Study the drawing (mm; zero at the part's minimum x, y, z) and answer. A direction names the side the tool comes from. Coordinates: 2 decimals unless noted, no trailing zeros. Order: outer loops, then holes, each group sorted by start corner. A loop starts at its lowest first (then second) coordinate and runs counter-clockwise, first axis right, second up. Notation, with made-up numbers: (53, 31.5) -> (90, 31.5) arc R21 cw to (90, 51.5) -> close; hole circle Ø11 at (69.25, 58). An arc over 180 degrees is marked (long way). Put each result on its own line as item: value. Start each with the question number.
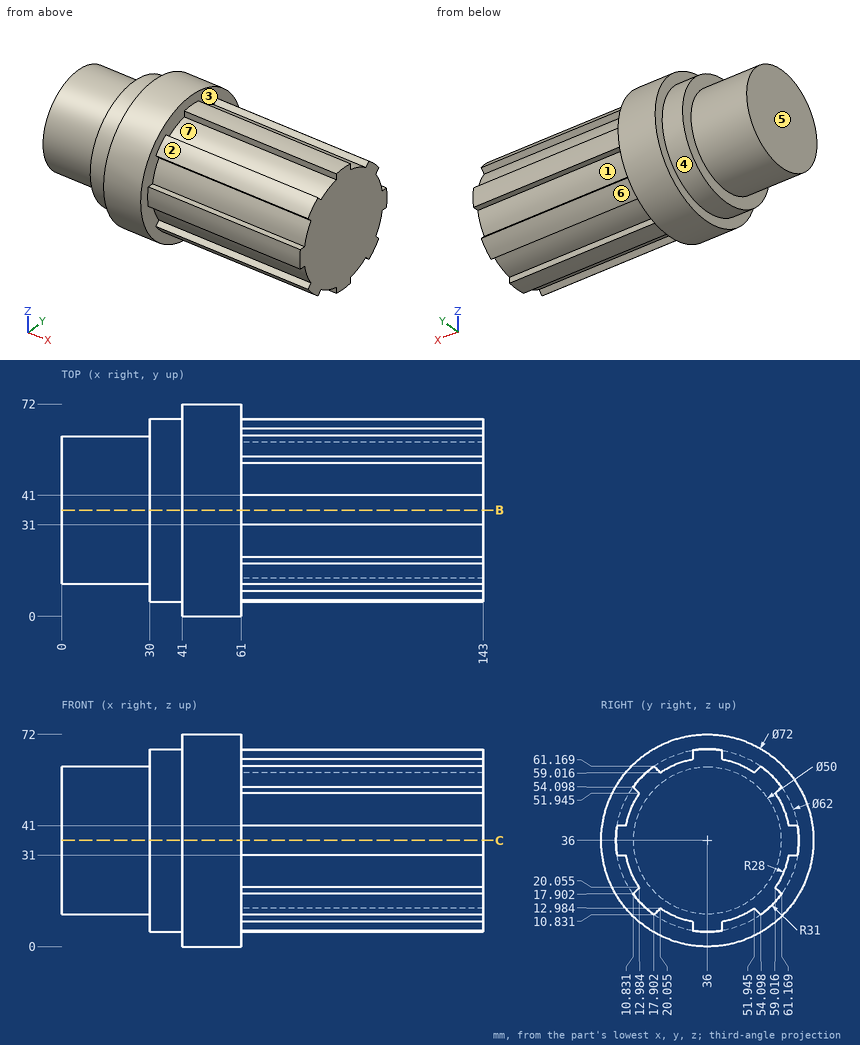
(1) For a pull along Y with two mould halves and no side action, classify the marked faces 5, 6 and 7 as released by +Y, released by -Y, zero draft, split by the parting line, or undercut.
(2) Each of these flat-tipped pins is pushed along its axis until it touches: P1, Ø0.9, axis at x = 83.5, z = 65, coming from the +Y side; P2, Ø1.5, axis at x = 101, y = 65, coming from the +Z side; P3, Ø3, axis at x = 36, y = 51.5, coming from the +Z side. Where does it stop, or does it pass through?
(3) The part is cut by section B-B on y = 36. Determine the outline of the cut face in (x, z).
(4) Find the intervals of material crossed by L1, parallel to Z at x = 86, y = 66.5; L2, parallel to Z at x = 77, y = 12.5 (1 decimal); L3, parallel to X at y = 8, z = 43, in increasing order.
(5) A tool of negligible diameter and unlimited length cuts with its end or side. For the marked faces 1, 2, 3 and 4, from which of +Z, -Z, +X, -X, +Y, -Y can it reach the whole face along a straight path? Write none if from no direction.
Worked out:
1. face 5: zero draft
1. face 6: released by +Y
1. face 7: undercut
2. P1: y = 41
2. P2: z = 41
2. P3: z = 63.66
3. outline: (0, 11) -> (30, 11) -> (30, 5) -> (41, 5) -> (41, 0) -> (61, 0) -> (61, 5) -> (143, 5) -> (143, 67) -> (61, 67) -> (61, 72) -> (41, 72) -> (41, 67) -> (30, 67) -> (30, 61) -> (0, 61) -> close
4. L1: 31 to 41
4. L2: 15.8 to 19.6, 20.8 to 51.2, 52.4 to 56.2
4. L3: 30 to 61
5. face 1: +X, +Y
5. face 2: +Z, +X, -Y
5. face 3: +X
5. face 4: -X
